Here's how the part is built. I have some questions about the finished solid (model axes, mm). Face numbers are marked on the shaded views. Coordinates: 2 decimals unless noted, no trailing zeros. Loops run counter-clockwise (first coordinate to the right, second up) from the corner with the lowest first, then second, coordinate; pieces in that order, holes last. Notation, with made-up numbers: (17, 87) -> (37, 87) arc R22 ccw to (37, 112) -> close; hole circle Ø7 at (3.25, 75). An arc over 180 degrees is marked (long way). Answer as a JSON object with one key per item and string values. Group by question number.
1) I need wall thicknesses on probe 1 along Y at (x, z) = (0, -3); probe 2 along X at (y, z) = (-5, -12.5); probe 3 along Y at (x, z) = (-2, -8). Which ranges of each line are inside material? Lowest first, please. Write a range as [from, to].
2) I want a section at C-C (z = 13.5). Write out the boundary of the cut face in (x, y), then the cut area to 3 significant figures.
3) I want a section at A-A (y = 0). Write out the boundary of the cut face in (x, z).
4) If we mould it in two halves opening along Y, with no side actions, what happens to the marked faces 1, 2 and 3? For each: +Y half, -Y half, draft (parallel to the pull), parting line (faces both ways), or undercut.
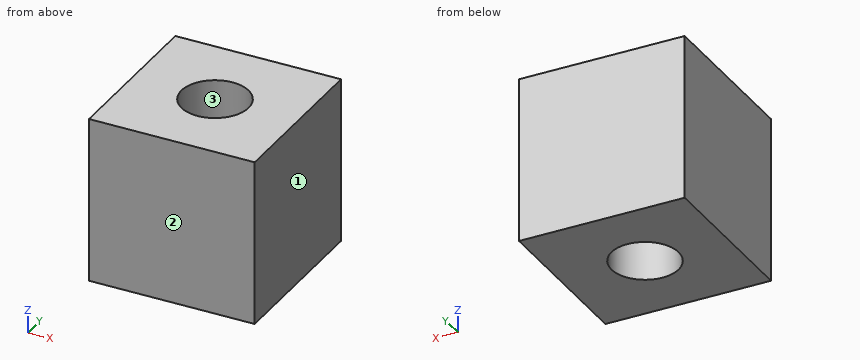
```python
from build123d import *

# Parameters (mm, degrees)
SKETCH_1_W          = 40
SKETCH_1_H          = 40
EXTRUDE_1_DEPTH     = 20
SKETCH_2_R          = 8.1
CUT_EXTRUDE_1_DEPTH = 40


with BuildPart() as part:
    # 草图1 → 凸台-拉伸1 (new, symmetric)
    with BuildSketch(Plane.XY):
        Rectangle(SKETCH_1_W, SKETCH_1_H)
    extrude(amount=EXTRUDE_1_DEPTH, both=True)

    # 草图2 → 切除-拉伸1 (cut, symmetric)
    with BuildSketch(Plane.XY):
        Circle(SKETCH_2_R)
    extrude(amount=CUT_EXTRUDE_1_DEPTH, both=True, mode=Mode.SUBTRACT)


solid = part.part
```
Determined:
{
 "1": {"probe 1": "[-20, -8.1], [8.1, 20]", "probe 2": "[-20, -6.37], [6.37, 20]", "probe 3": "[-20, -7.85], [7.85, 20]"},
 "2": {"outline": "(-20, -20) -> (20, -20) -> (20, 20) -> (-20, 20) -> close; hole circle Ø16.2 at (0, 0)", "area": "1,390 mm^2"},
 "3": {"outline": "(-20, -20) -> (-8.1, -20) -> (-8.1, 20) -> (-20, 20) -> close; (8.1, -20) -> (20, -20) -> (20, 20) -> (8.1, 20) -> close"},
 "4": {"face 1": "draft", "face 2": "-Y half", "face 3": "undercut"}
}
